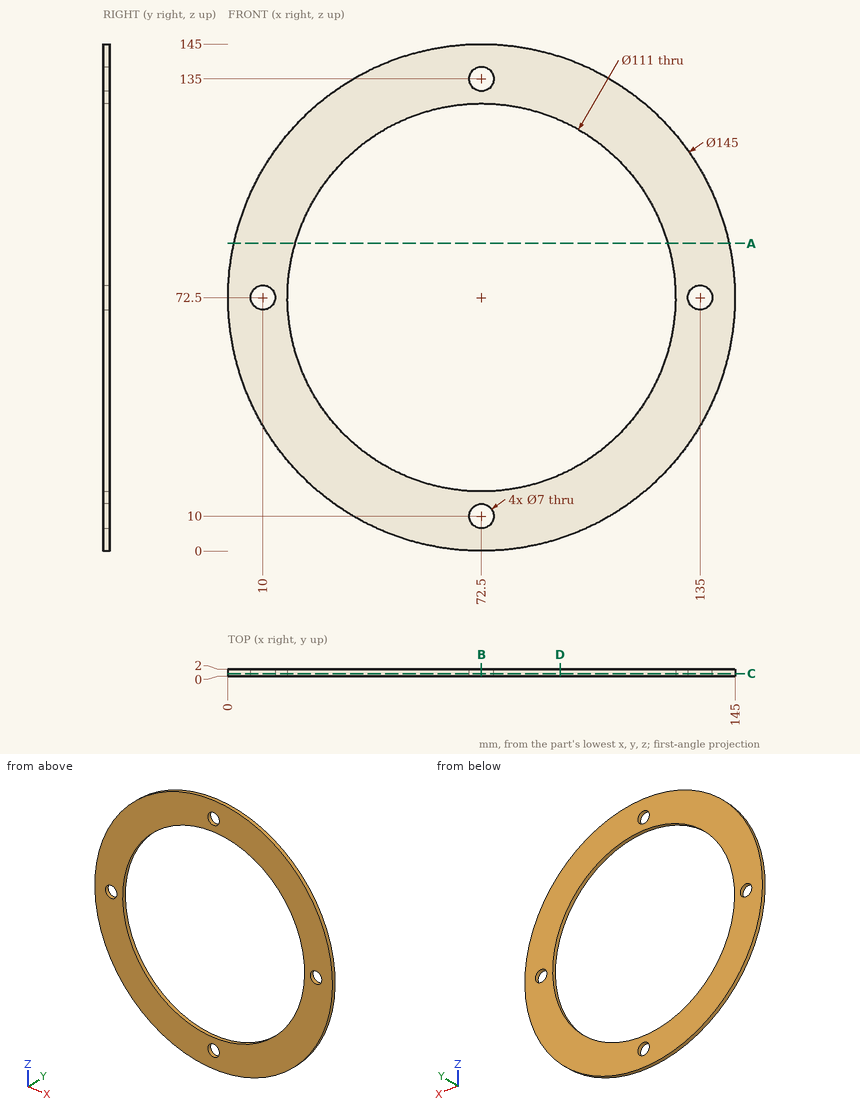
Job drawing, mm, ordinate dimensions from the low corner. One solid piece. Round coordinates to 2 decimals unless told otherwise and drop trailing zeros. Loops run counter-clockwise (first coordinate to the right, second up) from the corner with the lowest first, then second, coordinate; pieces in that order, holes last.
(1) Cut at B-B (x = 72.5). Give the cut face in (y, z), plus the area to 3 significant figures.
(2) Cut at A-A (z = 88). Give the cut face in (x, y).
(3) Drop a flat-ended pin along its axis: pin 1 (4 mm diameter, centred on x = 72.5, z = 10, fed in from -Y). Give the stop position or say it passes through.
(4) Cut at D-D (x = 95). Give the cut face in (y, z).
(5) Wall check: line 1 along Z through (x, y) = (31, 1.55); line 2 along Z through (x, y) = (74, 0.9); line 3 along X through (y, z) = (1.3, 10). Give the ranges that are in metal, low to high.
(6) Cut at C-C (y = 0.65). Give the cut face in (x, z), plus the area to 3 significant figures.
Findings below:
1. outline: (0, 0) - (2, 0) - (2, 6.5) - (0, 6.5) - close; (0, 13.5) - (2, 13.5) - (2, 17) - (0, 17) - close; (0, 128) - (2, 128) - (2, 131.5) - (0, 131.5) - close; (0, 138.5) - (2, 138.5) - (2, 145) - (0, 145) - close
1. area: 40.0 mm2
2. outline: (1.68, 0) - (19.21, 0) - (19.21, 2) - (1.68, 2) - close; (125.79, 0) - (143.32, 0) - (143.32, 2) - (125.79, 2) - close
3. pin 1: passes through
4. outline: (0, 3.58) - (2, 3.58) - (2, 21.77) - (0, 21.77) - close; (0, 123.23) - (2, 123.23) - (2, 141.42) - (0, 141.42) - close
5. line 1: z = 13.05 to 35.65, 109.35 to 131.95
5. line 2: z = 0.02 to 6.84, 13.16 to 17.02, 127.98 to 131.84, 138.16 to 144.98
5. line 3: x = 35.76 to 69, 76 to 109.24
6. outline: circle Ø145 at (72.5, 72.5); hole circle Ø7 at (10, 72.5); hole circle Ø111 at (72.5, 72.5); hole circle Ø7 at (72.5, 10); hole circle Ø7 at (72.5, 135); hole circle Ø7 at (135, 72.5)
6. area: 6,680 mm2
